Geometry check sheet. Reference: the model listing, model coordinates, mm. Face numbers are marked on the shaded views. A direction names the side the tool comes from. Round coordinates to 2 decimals unless told otherwise and drop trailing zeros. Order: outer loops, then holes, each group sorted by start corner. A loop starts at its lowest first (then second) coordinate and runs counter-clockwise, first axis right, second up.
(1) Sectioned sample at A-A (x = 0). Record the boundary of the cut face in (y, z), plus the area to 3 significant figures.
(2) Sectioned sample at B-B (y = 7). Record the boundary of the cut face in (x, z).
(3) Go/stop test with flat-tipped pins: pin 1 (1 mm diameter, centred on y = 12, z = 5, fed in from +X); pin 2 (16 mm diameter, centred on x = -44, z = 0, fed in from +Y); pin 3 (8 mm diameter, centred on y = 14.5, z = 25, fed in from -X); pin 4 (12 mm diameter, centred on x = 26, z = 10.5, fed in from -Y). Record where each tip stops, or that it passes through.
(4) Sectioned sample at C-C (z = 0). Record the boundary of the cut face in (x, y).
(5) Set-up check for the marked faces 5, 6 and 7: record each of +Z, -Z, +X, -X, +Y, -Y from which the full face is reachable in a straight line by a thin tool's end or side.
(6) Release check for a two-part mould opening along X. For the marked faces 1, 2, 3 and 4 record: +X half, -X half, draft (parallel to the pull), parting line (faces both ways), or undercut.
(7) Material ranges on line 1 along X through (y, z) = (2, -0.5); line 2 along Z through (x, y) = (3, 11.5); line 3 along Y through (x, z) = (3.5, 25), recorded low to high.
(8) Sectioned sample at D-D (z = 12.5). Record the boundary of the cut face in (x, y), plus the area to 3 significant figures.
from build123d import *

# Parameters (mm, degrees)
SKETCH_1_R          = 5
EXTRUDE_1_DEPTH     = 10
SKETCH_2_R          = 33
EXTRUDE_2_DEPTH     = 10
SKETCH_3_R          = 27.5
CUT_EXTRUDE_1_DEPTH = 15
SKETCH_4_R          = 24.5
CUT_EXTRUDE_2_DEPTH = 15


with BuildPart() as part:
    # 草图1 → 凸台-拉伸1 (new body)
    with BuildSketch(Plane(origin=(0, 0, 0), x_dir=(1, 0, 0), z_dir=(0, 1, 0))):
        with BuildLine():
            Line((-49.5, 9.526279442), (-16.5, 28.578838325))
            ThreePointArc((-16.5, 28.578838325), (0, 33), (16.5, 28.578838325))
            Line((16.5, 28.578838325), (49.5, 9.526279442))
            ThreePointArc((49.5, 9.526279442), (55, 0), (49.5, -9.526279442))
            Line((49.5, -9.526279442), (16.5, -28.578838325))
            ThreePointArc((16.5, -28.578838325), (0, -33), (-16.5, -28.578838325))
            Line((-16.5, -28.578838325), (-49.5, -9.526279442))
            ThreePointArc((-49.5, -9.526279442), (-55, 0), (-49.5, 9.526279442))
        make_face()
        with Locations(Location((-44, 0, 0), (0, 0, 270))):
            Circle(SKETCH_1_R, mode=Mode.SUBTRACT)
        with Locations(Location((44, 0, 0), (0, 0, 270))):
            Circle(SKETCH_1_R, mode=Mode.SUBTRACT)
    extrude(amount=EXTRUDE_1_DEPTH)

    # 草图2 → 凸台-拉伸2 (add)
    with BuildSketch(Plane(origin=(0, 10, 0), x_dir=(1, 0, 0), z_dir=(0, 1, 0))):
        with Locations(Location((0, 0, 0), (0, 0, 120))):
            Circle(SKETCH_2_R)
    extrude(amount=EXTRUDE_2_DEPTH)

    # 草图3 → 切除-拉伸1 (cut)
    with BuildSketch(Plane(origin=(0, 20, 0), x_dir=(1, 0, 0), z_dir=(0, 1, 0))):
        with Locations(Location((0, 0, 0), (0, 0, 270))):
            Circle(SKETCH_3_R)
    extrude(amount=-CUT_EXTRUDE_1_DEPTH, mode=Mode.SUBTRACT)

    # 草图4 → 切除-拉伸2 (cut)
    with BuildSketch(Plane(origin=(0, 5, 0), x_dir=(1, 0, 0), z_dir=(0, 1, 0))):
        with Locations(Location((0, 0, 0), (0, 0, 270))):
            Circle(SKETCH_4_R)
    extrude(amount=-CUT_EXTRUDE_2_DEPTH, mode=Mode.SUBTRACT)


solid = part.part
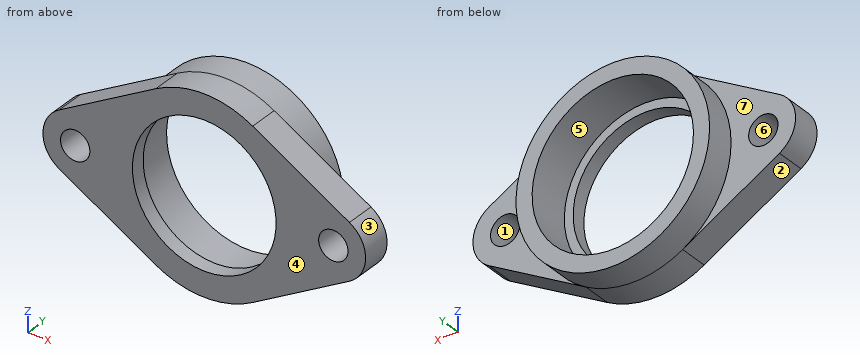
Answer below:
1. outline: (0, -33) - (20, -33) - (20, -27.5) - (5, -27.5) - (5, -24.5) - (0, -24.5) - close; (0, 24.5) - (5, 24.5) - (5, 27.5) - (20, 27.5) - (20, 33) - (0, 33) - close
1. area: 250 mm2
2. outline: (-49.5, -9.53) - (-16.5, -28.58) arc R33 ccw to (16.5, -28.58) - (49.5, -9.53) arc R11 ccw to (49.5, 9.53) - (16.5, 28.58) arc R33 ccw to (-16.5, 28.58) - (-49.5, 9.53) arc R11 ccw to start; hole circle Ø10 at (-44, 0); hole circle Ø55 at (0, 0); hole circle Ø10 at (44, 0)
3. pin 1: stops at x = 32.69
3. pin 2: stops at y = 10
3. pin 3: stops at x = -25.46
3. pin 4: stops at y = 0
4. outline: (-55, 0) - (-49, 0) - (-49, 10) - (-55, 10) - close; (-39, 0) - (-24.5, 0) - (-24.5, 5) - (-27.5, 5) - (-27.5, 20) - (-33, 20) - (-33, 10) - (-39, 10) - close; (24.5, 0) - (39, 0) - (39, 10) - (33, 10) - (33, 20) - (27.5, 20) - (27.5, 5) - (24.5, 5) - close; (49, 0) - (55, 0) - (55, 10) - (49, 10) - close
5. face 5: +Y
5. face 6: +Y, -Y
5. face 7: -X, +Y
6. face 1: undercut
6. face 2: -X half
6. face 3: +X half
6. face 4: draft
7. line 1: x = -54.99 to -48.97, -39.03 to -24.49, 24.49 to 39.03, 48.97 to 54.99
7. line 2: z = -32.86 to -27.34, 27.34 to 32.86
7. line 3: y = 0 to 5
8. outline: (-44.35, 0) - (-21.07, 0) - (-21.07, 5) - (-24.49, 5) - (-24.49, 20) - (-30.54, 20) - (-30.54, 10) - (-44.35, 10) - close; (21.07, 0) - (44.35, 0) - (44.35, 10) - (30.54, 10) - (30.54, 20) - (24.49, 20) - (24.49, 5) - (21.07, 5) - close
8. area: 552 mm2
